```python
from build123d import *

# Parameters (mm, degrees)
EXTRUDE_1_DEPTH         = 1170
HOLE_WIZARD_M10_1_D     = 8.5
HOLE_WIZARD_M10_1_DEPTH = 27.5
HOLE_WIZARD_M10_1_TIP   = 2.553657631


with BuildPart() as part:
    # 草图1 → 凸台-拉伸1 (new, symmetric)
    with BuildSketch(Plane.XY):
        Polygon((0, 0), (65, 0), (65, 4), (8.5, 8), (8.5, 152), (65, 156), (65, 160), (0, 160), align=None)
    extrude(amount=EXTRUDE_1_DEPTH, both=True)

    # M10 螺纹孔1
    with Locations(Plane.ZY):
        with Locations((-1010, 30), (610, 30), (-1010, 130), (610, 130)):
            Hole(HOLE_WIZARD_M10_1_D / 2, depth=HOLE_WIZARD_M10_1_DEPTH)
            with Locations((0, 0, -(HOLE_WIZARD_M10_1_DEPTH + HOLE_WIZARD_M10_1_TIP / 2))):  # 118° drill point
                Cone(0, HOLE_WIZARD_M10_1_D / 2, HOLE_WIZARD_M10_1_TIP, mode=Mode.SUBTRACT)


solid = part.part
```
Can you work these out from the model? Positions are in its coordinate system, mm. A direction names the side the tool comes from. Round coordinates to 2 decimals unless told otherwise and drop trailing zeros. Loops run counter-clockwise (first coordinate to the right, second up) from the corner with the lowest first, then second, coordinate; pieces in that order, holes last.
Item 1: If we mould it in two halves opening along Y, with no side actions, what happens to faces 3 (the flat face through (33, 160, 16)), 4 (the flat face through (0, 81, 16)), 5 (the flat face through (32, 0, 16)), 6 (the flat face through (8.5, 79, 16))? For each: +Y half, -Y half, draft (parallel to the pull), parting line (faces both ways), or undercut.
Item 2: Suppose I cut it at B-B, the plane z = -955. Write out the boundary of the cut face in (x, y).
Item 3: Suppose I cut it at C-C, the plane y = 92.5. Write out the boundary of the cut face in (x, z).
Item 4: Suppose I cut it at A-A, the plane x = 30. Write out the boundary of the cut face in (y, z).
Item 5: Which directions (+Z, -Z, +X, -X, +Y, -Y) give clear straight access to the entire face, cutting with the end or side of a thin tool? Please do faces 1 (the flat face through (8, 80, -1170)), 2 (the flat face through (37.15, 5.97, 16.38)).
Item 6: Will these pins go through, and if not, where does the flat tip stop? pin 1 Ø4 at (y, z) = (142.5, -644.5) entering from -X; pin 2 Ø1.5 at (y, z) = (125, 207) entering from +X.
Item 7: Please list where these lines run through material, in increasing order: L1, parallel to Y at x = 6.75, z = -1010; L2, parallel to Y at x = 13, z = 761.5; L3, parallel to Y at x = 14, z = 69.
Reported:
1. face 3: +Y half
1. face 4: draft
1. face 5: -Y half
1. face 6: undercut
2. outline: (0, 0) - (65, 0) - (65, 4) - (8.5, 8) - (8.5, 152) - (65, 156) - (65, 160) - (0, 160) - close
3. outline: (0, -1170) - (8.5, -1170) - (8.5, 1170) - (0, 1170) - close
4. outline: (0, -1170) - (6.48, -1170) - (6.48, 1170) - (0, 1170) - close; (153.52, -1170) - (160, -1170) - (160, 1170) - (153.52, 1170) - close
5. face 1: -Z, +X, -X, +Y, -Y
5. face 2: +Z, -Z, +X
6. pin 1: stops at x = 0
6. pin 2: stops at x = 8.5
7. L1: y = 0 to 25.75, 34.25 to 125.75, 134.25 to 160
7. L2: y = 0 to 7.68, 152.32 to 160
7. L3: y = 0 to 7.61, 152.39 to 160
